```python
from build123d import *

# Parameters (mm, degrees)
SKETCH1_R           = 35
SKETCH1_R_2         = 6.5
BOSS_EXTRUDE1_DEPTH = 2


with BuildPart() as part:
    # Sketch1 → Boss-Extrude1 (new, symmetric)
    with BuildSketch(Plane.XY):
        with BuildLine():
            ThreePointArc((30.608172596, 51.605617624), (0, 60), (-30.608172596, 51.605617624))
            ThreePointArc((-30.608172596, 51.605617624), (-50.204581464, 50.204581464), (-51.605617624, 30.608172596))
            ThreePointArc((-51.605617624, 30.608172596), (-60, 0), (-51.605617624, -30.608172596))
            ThreePointArc((-51.605617624, -30.608172596), (-50.204581464, -50.204581464), (-30.608172596, -51.605617624))
            ThreePointArc((-30.608172596, -51.605617624), (0, -60), (30.608172596, -51.605617624))
            ThreePointArc((30.608172596, -51.605617624), (50.204581464, -50.204581464), (51.605617624, -30.608172596))
            ThreePointArc((51.605617624, -30.608172596), (60, 0), (51.605617624, 30.608172596))
            ThreePointArc((51.605617624, 30.608172596), (50.204581464, 50.204581464), (30.608172596, 51.605617624))
        make_face()
        Circle(SKETCH1_R, mode=Mode.SUBTRACT)
        with Locations((39.597979746, 39.597979746)):
            Circle(SKETCH1_R_2, mode=Mode.SUBTRACT)
        with Locations((39.597979746, -39.597979746)):
            Circle(SKETCH1_R_2, mode=Mode.SUBTRACT)
        with Locations((-39.597979746, -39.597979746)):
            Circle(SKETCH1_R_2, mode=Mode.SUBTRACT)
        with Locations((-39.597979746, 39.597979746)):
            Circle(SKETCH1_R_2, mode=Mode.SUBTRACT)
    extrude(amount=BOSS_EXTRUDE1_DEPTH, both=True)


solid = part.part
```
The listing builds one solid part. Answer for the finished solid, in the listing's coordinates (mm). Round coordinates to 2 decimals unless told otherwise and drop trailing zeros. Write each loop counter-clockwise with the first axis right and the second up, starting at its lowest first coordinate (ties: lowest second). Pieces come first, ordered by that corner, then holes. Notation, with made-up numbers: (-3.75, -15.5) -> (28.25, -15.5) arc R26 ccw to (28.25, 6.5) -> close; hole circle Ø9 at (23.5, -14.75). An arc over 180 degrees is marked (long way). Write item = value, one per line.
1) For a pull along Y with two mould halves and no side action, classify faces 1 (the cylindrical face through (-44.389, -35.205, -0.028)), 2 (the cylindrical face through (-60, 0, 0)), 3 (the flat face through (26, -26, 2)), 4 (the cylindrical face through (0, 60, 0)) as released by +Y, released by -Y, zero draft, split by the parting line, or undercut.
Check values:
face_1 = undercut
face_2 = undercut
face_3 = zero draft
face_4 = released by +Y
2) Straight lines are drawn through the part: line 1 along X through (y, z) = (45, -0.3); line 2 along X through (y, z) = (0.5, -0.2); line 3 along X through (y, z) = (-52.5, 0.55). For each, find the intervals that lie inside material, in ascending order. Write a range as [from, to].
Check values:
line_1 = [-53.59, -43.21], [-35.98, 35.98], [43.21, 53.59]
line_2 = [-60, -35], [35, 60]
line_3 = [-47.25, -31.95], [-29.05, 29.05], [31.95, 47.25]
3) Section D-D on y = 42 is taken. Write down the section's boundary in (x, z).
Check values:
outline = (-54.4, -2) -> (-45.64, -2) -> (-45.64, 2) -> (-54.4, 2) -> close; (-33.56, -2) -> (33.56, -2) -> (33.56, 2) -> (-33.56, 2) -> close; (45.64, -2) -> (54.4, -2) -> (54.4, 2) -> (45.64, 2) -> close
4) Given pin 1 (21 mm diameter, centred on x = -39.6, y = 39.6, fed in from +Z); pin 2 (10.5 mm diameter, centred on x = 39.6, y = 39.6, fed in from -Z); pin 3 (1 mm diameter, centred on y = 40, z = 1, fed in from +X); pin 4 (1.5 mm diameter, centred on y = 6.5, z = 1, fed in from +X), each flat-ended and moving along its own axis, determine where each tip first touches the part or whether it passes through.
Check values:
pin_1 = 2
pin_2 = through
pin_3 = 54.6
pin_4 = 59.72
5) Section A-A on y = 0 is taken. Write down the section's boundary in (x, z), plus the area to 3 significant figures.
Check values:
outline = (-60, -2) -> (-35, -2) -> (-35, 2) -> (-60, 2) -> close; (35, -2) -> (60, -2) -> (60, 2) -> (35, 2) -> close
area = 200 mm²
6) Section C-C on z = -0.85 is taken. Write down the section's boundary in (x, y), plus the area to 3 significant figures.
Check values:
outline = (-51.61, -30.61) arc R15 ccw to (-30.61, -51.61) arc R60 ccw to (30.61, -51.61) arc R15 ccw to (51.61, -30.61) arc R60 ccw to (51.61, 30.61) arc R15 ccw to (30.61, 51.61) arc R60 ccw to (-30.61, 51.61) arc R15 ccw to (-51.61, 30.61) arc R60 ccw to start; hole circle Ø13 at (-39.6, -39.6); hole circle Ø13 at (-39.6, 39.6); hole circle Ø70 at (0, 0); hole circle Ø13 at (39.6, -39.6); hole circle Ø13 at (39.6, 39.6)
area = 7,940 mm²
